Here's the drawing with two shaded views (mm, measured from the low corner). I have some questions. Coordinates: 2 decimals unless noted, no trailing zeros. Order: outer loops, then holes, each group sorted by start corner. A loop starts at its lowest first (then second) coordinate and runs counter-clockwise, first axis right, second up. Notation, with made-up numbers: (75, 43.25) -> (103, 43.25) arc R19 cw to (103, 73.25) -> close; hole circle Ø10 at (58.5, 71.25). An arc over 180 degrees is marked (long way). Answer as a JSON object with one key per item and string values. Group by question number.
(1) For pin 1 (1 mm diameter, centred on y = 0.5, z = 18.5, fed in from -X) (3 decimals), with a flat end and sliding along its axis, tell me the tip position at first contact or that it passes through.
(2) I want a section at C-C, the plane x = 11.25. List the corners of the cut face in (y, z) for me, plus the area to 3 significant figures.
(3) I need wall thicknesses on line 1 (X direction, y = 1.1, z = 18.5); line 2 (X direction, y = 1.05, z = 12.5); line 3 (Z direction, x = 10.25, y = 0.65). Which ranges of each line are inside material? Lowest first, please.
(4) I want a section at A-A, the plane z = 12.5. List the corners of the cut face in (x, y) for me, plus the area to 3 significant figures.
(5) I want a section at B-B, the plane y = 1.1. List the corners of the cut face in (x, z) for me, plus the area to 3 significant figures.
(6) I want a section at D-D, the plane z = 6.5. List the corners of the cut face in (x, y) for me, plus the area to 3 significant figures.
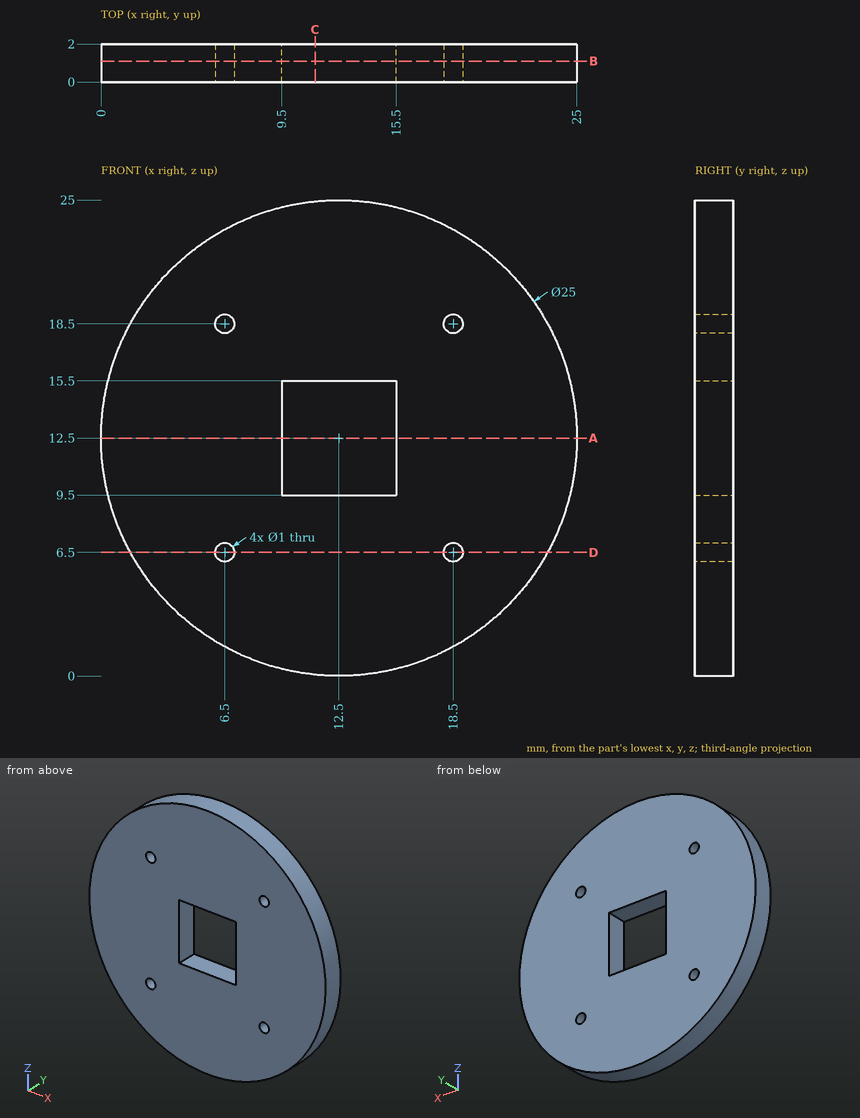
Computed values:
{
 "1": {"pin 1": "stops at x = 1.275"},
 "2": {"outline": "(0, 0.06) -> (2, 0.06) -> (2, 9.5) -> (0, 9.5) -> close; (0, 15.5) -> (2, 15.5) -> (2, 24.94) -> (0, 24.94) -> close", "area": "37.7 mm2"},
 "3": {"line 1": "x = 1.53 to 6, 7 to 18, 19 to 23.47", "line 2": "x = 0 to 9.5, 15.5 to 25", "line 3": "z = 0.2 to 9.5, 15.5 to 24.8"},
 "4": {"outline": "(0, 0) -> (9.5, 0) -> (9.5, 2) -> (0, 2) -> close; (15.5, 0) -> (25, 0) -> (25, 2) -> (15.5, 2) -> close", "area": "38.0 mm2"},
 "5": {"outline": "circle Ø25 at (12.5, 12.5); hole circle Ø1 at (6.5, 6.5); hole circle Ø1 at (6.5, 18.5); hole (9.5, 9.5) -> (15.5, 9.5) -> (15.5, 15.5) -> (9.5, 15.5) -> close; hole circle Ø1 at (18.5, 6.5); hole circle Ø1 at (18.5, 18.5)", "area": "452 mm2"},
 "6": {"outline": "(1.53, 0) -> (6, 0) -> (6, 2) -> (1.53, 2) -> close; (7, 0) -> (18, 0) -> (18, 2) -> (7, 2) -> close; (19, 0) -> (23.47, 0) -> (23.47, 2) -> (19, 2) -> close", "area": "39.9 mm2"}
}
